```python
from build123d import *

# Parameters (mm, degrees)
BOSS_EXTRUDE1_DEPTH = 102


with BuildPart() as part:
    # Sketch1 → Boss-Extrude1 (new body)
    with BuildSketch(Plane.XY):
        Polygon((0, 0), (0, 5), (-15, 12), (-70, 12), (-70, 0), align=None)
    extrude(amount=BOSS_EXTRUDE1_DEPTH)


solid = part.part
```
Part model, mm, in its own coordinate system. Coordinates: 2 decimals unless noted, no trailing zeros. Order: outer loops, then holes, each group sorted by start corner. A loop starts at its lowest first (then second) coordinate and runs counter-clockwise, first axis right, second up. Notation, with made-up numbers: (46, 54.5) - (58, 54.5) arc R20 ccw to (58, 76.5) - close; hole circle Ø5 at (46.5, 81). An arc over 180 degrees is marked (long way). Return JSON: item names as keys, results as strings. Group by question number.
Item 1: Drill centre lines: probe 1 along Y at (x, z) = (-10, 30.5); probe 2 along X at (y, z) = (10.5, 94); probe 3 along X at (y, z) = (9.75, 80). Where is each one in solid material? Low to high. Write a range as from..to.
Item 2: Cut at A-A (z = 94). List the corners of the cut face in (x, y), plus the area to 4 significant figures.
Item 3: Pin check, flat tips, straight feed: pin 1 (4 mm diameter, centred on y = 10, z = 81, fed in from +X); pin 2 (1 mm diameter, centred on x = -13.5, z = 60.5, fed in from +Y); pin 3 (2 mm diameter, centred on y = 8.5, z = 39, fed in from +X). Stop position of each tip, or through.
Item 4: Cut at B-B (y = 10). List the corners of the cut face in (x, z).
Check values:
{
 "1": {"probe 1": "y = 0..9.67", "probe 2": "x = -70..-11.79", "probe 3": "x = -70..-10.18"},
 "2": {"outline": "(-70, 0) - (0, 0) - (0, 5) - (-15, 12) - (-70, 12) - close", "area": "787.5 mm2"},
 "3": {"pin 1": "stops at x = -6.43", "pin 2": "stops at y = 11.53", "pin 3": "stops at x = -5.36"},
 "4": {"outline": "(-70, 0) - (-10.71, 0) - (-10.71, 102) - (-70, 102) - close"}
}
